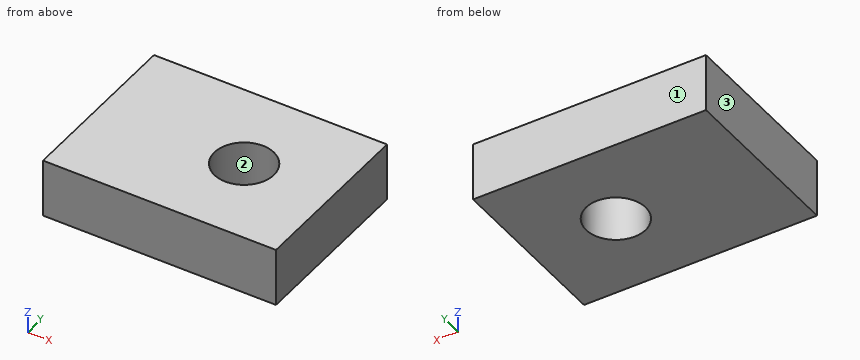
```python
from build123d import *

# Parameters (mm, degrees)
SKETCH1_W           = 40
SKETCH1_H           = 30
SKETCH1_R           = 5
BOSS_EXTRUDE1_DEPTH = 10
M12_TAPPED_HOLE1_D  = 10.2


with BuildPart() as part:
    # Sketch1 → Boss-Extrude1 (new body)
    with BuildSketch(Plane.XY):
        Rectangle(SKETCH1_W, SKETCH1_H)
        with Locations((5, 0)):
            Circle(SKETCH1_R, mode=Mode.SUBTRACT)
    extrude(amount=BOSS_EXTRUDE1_DEPTH)

    # M12 Tapped Hole1 (through all)
    with Locations(Plane(origin=(5, 0, 0), x_dir=(-1, 0, 0), z_dir=(0, 0, -1))):
        with Locations((0, 0)):
            Hole(M12_TAPPED_HOLE1_D / 2)


solid = part.part
```
Work out the finished part from the listing and answer in its coordinate system (mm). Face numbers are marked on the shaded views. Give positions to 0.01 mm unless a question says otherwise; leave off trailing zeros. Order: outer loops, then holes, each group sorted by start corner. A loop starts at its lowest first (then second) coordinate and runs counter-clockwise, first axis right, second up. Notation, with made-up numbers: M 49.25,70.5 L 96.25,70.5 A21 ccw 96.25,97.5 Z; hole C -10,40.25 d11. An arc over 180 degrees is marked long. Return JSON: item names as keys, results as strings.
1) Section C-C, the plane z = 2 is taken. Write down the section's boundary in (x, y), plus the area to 3 significant figures.
Resolved:
{"outline": "M -20,-15 L 20,-15 L 20,15 L -20,15 Z; hole C 5,0 d10.2", "area": "1,120 mm^2"}
2) Section A-A, the plane y = -4.5 is taken. Write down the section's boundary in (x, z), plus the area to 3 significant figures.
Resolved:
{"outline": "M -20,0 L 2.6,0 L 2.6,10 L -20,10 Z; M 7.4,0 L 20,0 L 20,10 L 7.4,10 Z", "area": "352 mm^2"}
3) For a pull along X with two mould halves and no side action, classify the marked faces 1, 2 and 3 as +X half, -X half, draft (parallel to the pull), parting line (faces both ways), or undercut.
Resolved:
{"face 1": "draft", "face 2": "undercut", "face 3": "-X half"}
4) Section B-B, the plane x = 5 is taken. Write down the section's boundary in (y, z).
Resolved:
{"outline": "M -15,0 L -5.1,0 L -5.1,10 L -15,10 Z; M 5.1,0 L 15,0 L 15,10 L 5.1,10 Z"}
5) Straight lines are drawn through the part: line 1 along Y through (x, z) = (5, 6.5); line 2 along Y through (x, z) = (7, 7.5); line 3 along X through (y, z) = (4, 4). For each, find the intervals that lie inside material, in ascending order. Write a range as [from, to].
Resolved:
{"line 1": "[-15, -5.1], [5.1, 15]", "line 2": "[-15, -4.69], [4.69, 15]", "line 3": "[-20, 1.84], [8.16, 20]"}
